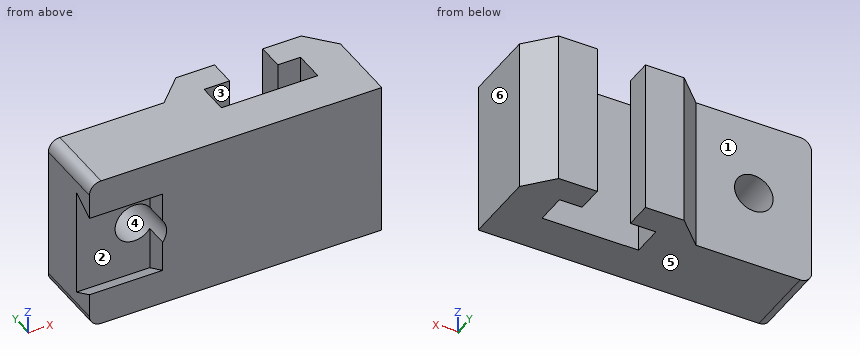
```python
from build123d import *

# Parameters (mm, degrees)
BASE_BODY_DEPTH    = 80
RAISED_BLOCK_DEPTH = 38
WEDGE_BOSS_DEPTH   = 80
TOP_HOLE_SKETCH_R  = 10
TOP_HOLE_DEPTH     = 38
PROFILE_CUT_DEPTH  = 38


with BuildPart() as part:
    # Base Profile Sketch → Base Body (new body)
    with BuildSketch(Plane.XY):
        with BuildLine():
            Line((52.5, 0), (54, 0))
            Line((54, 0), (144, 0))
            Line((144, 0), (144, 22))
            Line((144, 22), (144, 38))
            Line((144, 38), (131.5, 52))
            Line((131.5, 52), (111.5, 52))
            Line((111.5, 52), (111.5, 38))
            Line((111.5, 38), (123.25, 38))
            Line((123.25, 38), (123.25, 22))
            Line((123.25, 22), (73.25, 22))
            Line((73.25, 22), (73.25, 38))
            Line((73.25, 38), (86.5, 38))
            Line((86.5, 38), (86.5, 52))
            Line((86.5, 52), (66.5, 52))
            Line((66.5, 52), (52.5, 38))
            Line((52.5, 38), (-1.5, 38))
            Line((-1.5, 38), (-1.5, 0))
            ThreePointArc((-1.5, 0), (-0.743974245, 0.047821822), (0, 0.190524981))
            Line((0, 0.190524981), (0, 0))
            Line((0, 0), (52.5, 0))
        make_face()
    extrude(amount=BASE_BODY_DEPTH)

    # Raised Block Sketch → Raised Block (add)
    with BuildSketch(Plane(origin=(0, 38, 0), x_dir=(1, 0, 0), z_dir=(0, 1, 0))):
        with BuildLine():
            Line((-1.5, 0), (-1.5, -6))
            Line((-1.5, -6), (-1.5, -74))
            Line((-1.5, -74), (-1.5, -80))
            ThreePointArc((-1.5, -80), (-5.742640687, -78.242640687), (-7.5, -74))
            Line((-7.5, -74), (-7.5, -6))
            ThreePointArc((-7.5, -6), (-5.742640687, -1.757359313), (-1.5, 0))
        make_face()
    extrude(amount=-RAISED_BLOCK_DEPTH)

    # Wedge Sketch → Wedge Boss (add)
    with BuildSketch(Plane(origin=(0, 0, 0), x_dir=(-1, 0, 0), z_dir=(0, 0, -1))):
        Polygon((0, 0.190524981), (0, 0), (1.5, 0), align=None)
    extrude(amount=-WEDGE_BOSS_DEPTH)

    # Top Hole Sketch → Top Hole (cut)
    with BuildSketch(Plane(origin=(0, 38, 0), x_dir=(1, 0, 0), z_dir=(0, 1, 0))):
        with Locations(Location((22.5, -40, 0), (0, 0, 270))):
            Circle(TOP_HOLE_SKETCH_R)
    extrude(amount=-TOP_HOLE_DEPTH, mode=Mode.SUBTRACT)

    # Profile Cut Sketch → Profile Cut (cut)
    with BuildSketch(Plane.ZY.offset(7.5)):
        Polygon((68, 11.989734921), (40, 11.989734921), (12, 11.989734921), (18.2, 0), (40, 0), (61.077723316, 0), align=None)
    extrude(amount=-PROFILE_CUT_DEPTH, mode=Mode.SUBTRACT)


solid = part.part
```
Check sheet for the modelled part. Datum: model origin and axes. Units: mm. Face numbers are marked on the shaded views. A direction names the side the tool comes from. Give positions to 0.01 mm unless a question says otherwise; leave off trailing zeros. Write each loop counter-clockwise with the first axis right and the second up, starting at its lowest first coordinate (ties: lowest second). Pieces come first, ordered by that corner, then holes. Notation, with made-up numbers: (-4, 59.5) -> (11, 59.5) arc R16 ccw to (11, 80.5) -> close; hole circle Ø5 at (85, 2). An arc over 180 degrees is marked (long way). Use CSV: the item, a comma, the result in double quotes. Start each with the question number.
Q1. Cross-section at B-B on y = 33.5. Enter the section's corners in (x, z).
Q2. Scan lines: line 1 along X through (y, z) = (26, 40); line 2 along X through (y, z) = (29, 56.5); line 3 along Z through (x, y) = (22, 18). Record each from-to range of solid material in increasing order.
Q3. Depth check by flat-ended pin: P1, Ø8, axis at y = 43.5, z = 14.5, coming from the +X side; P2, Ø7, axis at y = 43.5, z = 37, coming from the -X side; P3, Ø6, axis at y = 8, z = 58.5, coming from the -X side. Enter the tip coordinate at first touch or a pass-through.
Q4. Tool access check on the marked faces 1, 2 and 3. Record the directions out of +Z, -Z, +X, -X, +Y, -Y that give a thin tool (end or side, any length) a straight path to the whole face; none if there is none.
Q5. Cross-section at A-A on x = 79. Enter the section's corners in (y, z), and give its area (3 significant figures).
Q6. Cross-section at C-C on z = 40. Enter the section's corners in (x, y), and give its area (3 significant figures).
Q7. Release check for a two-part mould opening along Z. For the marked faces 4, 5 and 6 record: +Z half, -Z half, draft (parallel to the pull), parting line (faces both ways), or undercut.
Q8. Cross-section at D-D on y = 16.5. Enter the section's corners in (x, z).
Working result:
1,outline,"(-7.5, 6) arc R6 ccw to (-1.5, 0) -> (73.25, 0) -> (73.25, 80) -> (-1.5, 80) arc R6 ccw to (-7.5, 74) -> close; (123.25, 0) -> (144, 0) -> (144, 80) -> (123.25, 80) -> close; hole circle Ø20 at (22.5, 40)"
2,line 1,"x = -7.5 to 12.5, 32.5 to 73.25, 123.25 to 144"
2,line 2,"x = -7.5 to 73.25, 123.25 to 144"
2,line 3,"z = 0 to 30.01, 49.99 to 80"
3,P1,"stops at x = 142.66"
3,P2,"stops at x = 54.5"
3,P3,"stops at x = 30.5"
4,face 1,"+Z, -Z, -X, +Y"
4,face 2,"-X"
4,face 3,"+Z, -Z"
5,outline,"(0, 0) -> (22, 0) -> (22, 80) -> (0, 80) -> close; (38, 0) -> (52, 0) -> (52, 80) -> (38, 80) -> close"
5,area,"2,880 mm^2"
6,outline,"(-7.5, 11.99) -> (12.5, 11.99) -> (12.5, 38) -> (-7.5, 38) -> close; (32.5, 0) -> (144, 0) -> (144, 38) -> (131.5, 52) -> (111.5, 52) -> (111.5, 38) -> (123.25, 38) -> (123.25, 22) -> (73.25, 22) -> (73.25, 38) -> (86.5, 38) -> (86.5, 52) -> (66.5, 52) -> (52.5, 38) -> (32.5, 38) -> close"
6,area,"4,700 mm^2"
7,face 4,"undercut"
7,face 5,"-Z half"
7,face 6,"draft"
8,outline,"(-7.5, 6) arc R6 ccw to (-1.5, 0) -> (144, 0) -> (144, 80) -> (-1.5, 80) arc R6 ccw to (-7.5, 74) -> close; hole circle Ø20 at (22.5, 40)"
